```python
from build123d import *

# Parameters (mm, degrees)
SKETCH1_R           = 5
BOSS_EXTRUDE1_DEPTH = 45
SKETCH2_R           = 6.5
BOSS_EXTRUDE2_DEPTH = 3
CHAMFER1_SIZE       = 0.5


with BuildPart() as part:
    # Sketch1 → Boss-Extrude1 (new body)
    with BuildSketch(Plane.XY):
        with Locations(Location((0, 0, 0), (0, 0, 180))):
            Circle(SKETCH1_R)
    extrude(amount=BOSS_EXTRUDE1_DEPTH)

    # Sketch2 → Boss-Extrude2 (add)
    with BuildSketch(Plane.XY.offset(45)):
        Circle(SKETCH2_R)
    extrude(amount=BOSS_EXTRUDE2_DEPTH)

    # Chamfer1
    chamfer1_edges = [part.edges().sort_by_distance(p)[0] for p in [
        (5, 0, 0),
        (-6.5, 0, 45),
        (-6.5, 0, 48),
    ]]
    chamfer(chamfer1_edges, length=CHAMFER1_SIZE)


solid = part.part
```
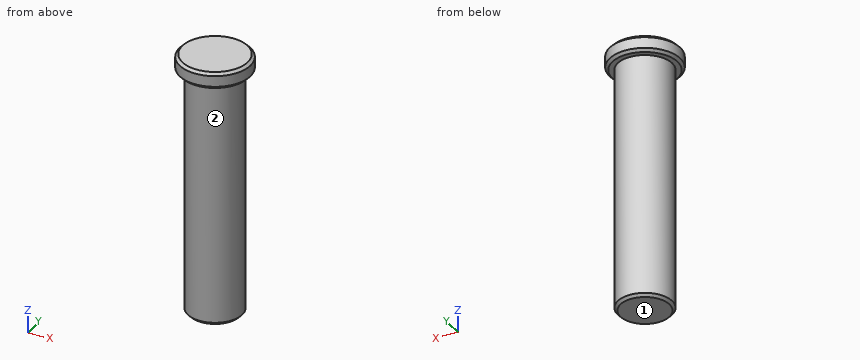
Geometry check sheet. Reference: the model listing, model coordinates, mm. Face numbers are marked on the shaded views. A direction names the side the tool comes from. Round coordinates to 2 decimals unless told otherwise and drop trailing zeros. Write each loop counter-clockwise with the first axis right and the second up, starting at its lowest first coordinate (ties: lowest second). Pieces come first, ordered by that corner, then holes. Notation, with made-up numbers: (-17, 66) -> (7, 66) arc R24 ccw to (7, 99) -> close; hole circle Ø4 at (-16, -16). An arc over 180 degrees is marked (long way). Put each result on its own line as item: value.
1) Depth check by flat-ended pin: P1, Ø3, axis at x = 1.5, z = 23, coming from the -Y side; P2, Ø1, axis at y = 3, z = 43, coming from the +X side; P3, Ø5, axis at y = -4.5, z = 20, coming from the +X side. Enter the tip coordinate at first touch or a pass-through.
Recorded:
P1: stops at y = -5
P2: stops at x = 4.33
P3: stops at x = 4.58
2) Cross-section at A-A, the plane y = 0. Enter the section's corners in (x, z), plus the area to 3 significant figures.
Recorded:
outline: (-6.5, 45.5) -> (-6, 45) -> (-5, 45) -> (-5, 0.5) -> (-4.5, 0) -> (4.5, 0) -> (5, 0.5) -> (5, 45) -> (6, 45) -> (6.5, 45.5) -> (6.5, 47.5) -> (6, 48) -> (-6, 48) -> (-6.5, 47.5) -> close
area: 488 mm2
3) Thickness scan on probe 1 along X at (y, z) = (0.25, 41); probe 2 along Z at (x, y) = (-5.25, 1.5). Record the ranges inside material, lowest first. Write a range as from..to.
Recorded:
probe 1: x = -4.99..4.99
probe 2: z = 45..48
4) Access from +Z, -Z, +X, -X, +Y, -Y to the whole of each face (thin tool, end or side, straight path). Record for the marked faces 1 and 2.
Recorded:
face 1: -Z, +X, -X, +Y, -Y
face 2: -Z
5) Cross-section at C-C, the plane z = 38. Enter the section's corners in (x, y), plus the area to 3 significant figures.
Recorded:
outline: circle Ø10 at (0, 0)
area: 78.5 mm2
